from build123d import *

# Parameters (mm, degrees)
SKETCH1_R           = 7.5
SKETCH1_R_2         = 3
BOSS_EXTRUDE1_DEPTH = 23
BOSS_EXTRUDE2_START = -10
SKETCH2_R           = 14
SKETCH2_R_2         = 3
BOSS_EXTRUDE2_DEPTH = 10
CHAMFER1_SIZE       = 1
SKETCH3_R           = 2
CUT_EXTRUDE1_DEPTH  = 15


with BuildPart() as part:
    # Sketch1 → Boss-Extrude1 (new body)
    with BuildSketch(Plane(origin=(0, 0, 0), x_dir=(1, 0, 0), z_dir=(0, 1, 0))):
        with Locations(Location((0, 0, 0), (0, 0, 270))):
            Circle(SKETCH1_R)
        with Locations(Location((0, 0, 0), (0, 0, 270))):
            Circle(SKETCH1_R_2, mode=Mode.SUBTRACT)
    extrude(amount=BOSS_EXTRUDE1_DEPTH)

    # Sketch2 → Boss-Extrude2 (add)
    with BuildSketch(Plane(origin=(0, 23, 0), x_dir=(1, 0, 0), z_dir=(0, 1, 0)).offset(BOSS_EXTRUDE2_START)):
        with Locations(Location((0, 0, 0), (0, 0, 270))):
            Circle(SKETCH2_R)
        with Locations(Location((0, 0, 0), (0, 0, 270))):
            Circle(SKETCH2_R_2, mode=Mode.SUBTRACT)
    extrude(amount=BOSS_EXTRUDE2_DEPTH)

    # Chamfer1
    chamfer1_edges = [part.edges().sort_by_distance(p)[0] for p in [
        (0, 23, -14),
        (0, 13, -14),
        (0, 0, -7.5),
    ]]
    chamfer(chamfer1_edges, length=CHAMFER1_SIZE)

    # Sketch3 → Cut-Extrude1 (cut)
    with BuildSketch(Plane(origin=(0, 0, 0), x_dir=(0, 0, -1), z_dir=(1, 0, 0))):
        with Locations((0, 7.039629159)):
            Circle(SKETCH3_R)
    extrude(amount=-CUT_EXTRUDE1_DEPTH, mode=Mode.SUBTRACT)


solid = part.part
For this review, take the finished solid that the model builds, in its own axes (mm). A direction names the side the tool comes from. Round coordinates to 2 decimals unless told otherwise and drop trailing zeros. Order: outer loops, then holes, each group sorted by start corner. A loop starts at its lowest first (then second) coordinate and runs counter-clockwise, first axis right, second up. Notation, with made-up numbers: M 73.5,63 L 92.5,63 A26 cw 92.5,95 Z; hole C 44.25,57.5 d1. An arc over 180 degrees is marked long. Use a Markdown table: item, result. Add a question column.
Item 1: To check wall thickness, follow line 1 along Y through (x, z) = (-3.65, 0); line 2 along X through (y, z) = (15.75, 0); line 3 along X through (y, z) = (1.25, 2.25). State the ranges of each line that lie inside material, in increasing order.
Item 2: Add section B-B, the plane x = 0. Give the boundary of the cut face in (y, z), then the cut area to 3 significant figures.
Item 3: Tool access review of faces 1 (the flat face through (-6, 13, 6)), 2 (the flat face through (-3, 23, 3)), 3 (the cylindrical face through (-4.835, 6.274, -1.847)): name each direction out of +Z, -Z, +X, -X, +Y, -Y from which nothing blocks a thin tool from reaching the whole face with its end or side.
Item 4: Mouldability with a two-part tool opening along Z and no side actions: class faces 4 (the flat face through (-1, 0, 3)), 5 (the cylindrical face through (-13.67, 17.94, -3.03)), 6 (the cylindrical face through (3, 11, 0)) as released by +Z, released by -Z, zero draft, split by the parting line, or undercut.
Item 5: Insertion check: pin 1 (12 mm diameter, centred on y = 8, z = 3.5, fed in from -X); pin 2 (1.5 mm diameter, centred on y = 4, z = 3.5, fed in from -X); pin 3 (1 mm diameter, centred on y = 6.5, z = -7, fed in from -X); pin 4 (10 mm diameter, centred on x = -3.5, y = 15.5, fed in from -Z). Each pin has a flat end and moves straight along its axis. Give the tip position at first contact, or say it passes through.
Item 6: Add section A-A, the plane z = 0. Give the boundary of the cut face in (x, y), then the cut area to 3 significant figures.
Item 7: Add section C-C, the plane y = 20.25. Give the boundary of the cut face in (x, z), then the cut area to 3 significant figures.
Geometry results:
| question | item | result |
|---|---|---|
| 1 | line 1 | y = 0 to 5.04, 9.04 to 23 |
| 1 | line 2 | x = -14 to -3, 3 to 14 |
| 1 | line 3 | x = -7.15 to -1.98, 1.98 to 7.15 |
| 2 | outline | M 0,-6.5 L 1,-7.5 L 13,-7.5 L 13,-13 L 14,-14 L 22,-14 L 23,-13 L 23,-3 L 0,-3 Z; M 0,3 L 23,3 L 23,13 L 22,14 L 14,14 L 13,13 L 13,7.5 L 1,7.5 L 0,6.5 Z |
| 2 | area | 334 mm² |
| 3 | face 1 | -Y |
| 3 | face 2 | +Z, -Z, +X, -X, +Y |
| 3 | face 3 | -X |
| 4 | face 4 | zero draft |
| 4 | face 5 | split by the parting line |
| 4 | face 6 | undercut |
| 5 | pin 1 | stops at x = -13.69 |
| 5 | pin 2 | stops at x = -6.98 |
| 5 | pin 3 | stops at x = -3.74 |
| 5 | pin 4 | stops at z = -14 |
| 6 | outline | M -14,14 L -13,13 L -7.5,13 L -7.5,9.04 L -3,9.04 L -3,23 L -13,23 L -14,22 Z; M -7.5,1 L -6.5,0 L -3,0 L -3,5.04 L -7.5,5.04 Z; M 3,0 L 6.5,0 L 7.5,1 L 7.5,13 L 13,13 L 14,14 L 14,22 L 13,23 L 3,23 Z |
| 6 | area | 316 mm² |
| 7 | outline | C 0,0 d28; hole C 0,0 d6 |
| 7 | area | 587 mm² |
